from build123d import *

# Parameters (mm, degrees)
SKETCH_2_W          = 165
SKETCH_2_H          = 130
EXTRUDE_1_DEPTH     = 10
SKETCH_3_W          = 116
SKETCH_3_H          = 10
CUT_EXTRUDE_1_DEPTH = 10
CUT_EXTRUDE_2_DEPTH = 106.50473923
CHAMFER_1_SIZE      = 35
HOLE_WIZARD_M6_1_D  = 5
CHAMFER_3_SIZE      = 3


with BuildPart() as part:
    # 草图2 → 凸台-拉伸1 (new body)
    with BuildSketch(Plane(origin=(0, 0, 0), x_dir=(1, 0, 0), z_dir=(0, 1, 0))):
        Rectangle(SKETCH_2_W, SKETCH_2_H)
    extrude(amount=EXTRUDE_1_DEPTH)

    # 草图3 → 切除-拉伸1 (cut)
    with BuildSketch(Plane(origin=(0, 10, 0), x_dir=(1, 0, 0), z_dir=(0, 1, 0))):
        with Locations((0, 60)):
            Rectangle(SKETCH_3_W, SKETCH_3_H)
    extrude(amount=-CUT_EXTRUDE_1_DEPTH, mode=Mode.SUBTRACT)

    # 草图4 → 切除-拉伸2 (cut, through all)
    with BuildSketch(Plane(origin=(0, 10, 0), x_dir=(1, 0, 0), z_dir=(0, 1, 0))):
        with BuildLine():
            Line((75, 57.5), (75, 32.5))
            ThreePointArc((75, 32.5), (70.5, 28), (66, 32.5))
            Line((66, 32.5), (66, 57.5))
            ThreePointArc((66, 57.5), (70.5, 62), (75, 57.5))
        make_face()
        with BuildLine():
            Line((75, 17.5), (75, -7.5))
            ThreePointArc((75, -7.5), (70.5, -12), (66, -7.5))
            Line((66, -7.5), (66, 17.5))
            ThreePointArc((66, 17.5), (70.5, 22), (75, 17.5))
        make_face()
    cut_extrude_2 = extrude(amount=-CUT_EXTRUDE_2_DEPTH, mode=Mode.SUBTRACT)

    # 倒角1
    chamfer_1_edges = [part.edges().sort_by_distance(p)[0] for p in [
        (82.5, 5, 65),
        (-82.5, 5, 65),
    ]]
    chamfer(chamfer_1_edges, length=CHAMFER_1_SIZE)

    # M6 螺纹孔1 (through all)
    with Locations(Plane(origin=(0, 10, 0), x_dir=(1, 0, 0), z_dir=(0, 1, 0))):
        with Locations((21, -14), (21, 34), (-21, 34), (-21, -14)):
            Hole(HOLE_WIZARD_M6_1_D / 2)

    # 倒角3
    chamfer_3_edges = [part.edges().sort_by_distance(p)[0] for p in [
        (-82.5, 5, -65),
        (82.5, 5, -65),
    ]]
    chamfer(chamfer_3_edges, length=CHAMFER_3_SIZE)

    # 镜向1: 切除-拉伸2 across plane
    add(cut_extrude_2.mirror(Plane(origin=(0, 0, 0), x_dir=(0, 0, 1), z_dir=(1, 0, 0))), mode=Mode.SUBTRACT)


solid = part.part
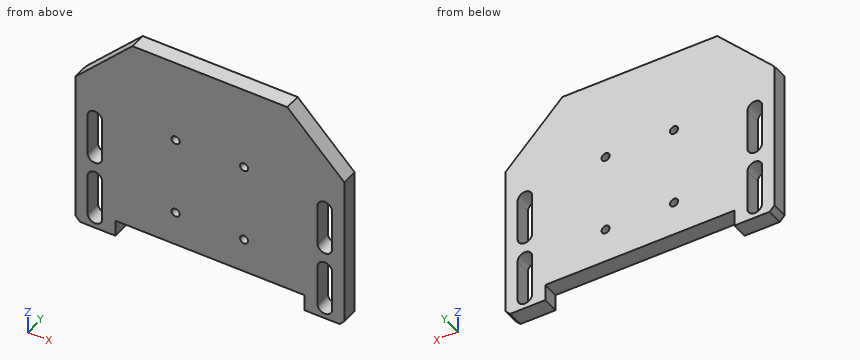
Work out the finished part from the listing and answer in its coordinate system (mm). Coordinates: 2 decimals unless noted, no trailing zeros. Loops run counter-clockwise (first coordinate to the right, second up) from the corner with the lowest first, then second, coordinate; pieces in that order, holes last. Notation, with made-up numbers: (13, 87.5) -> (68, 87.5) arc R11 cw to (68, 94.5) -> close; hole circle Ø4 at (-19.5, -1). An arc over 180 degrees is marked (long way). Write each question's results on one line, items separated by ' | '. Start each with the question number.
1) Find section C-C on y = 1.75. Count the separate pieces of the cut face and the enclosed holes in it, then the cut area to 3 significant figures.
2) Find section A-A on z = -5.5. Determine the outline of the cut face in (x, y).
3) Find section D-D on z = 37. Determine the outline of the cut face in (x, y), then the cut area to 3 significant figures.
4) Flat-ended cylindrical pins translate along their axes: P1, Ø6, axis at x = 21, z = 14, coming from the -Y side; P2, Ø6, axis at y = 6.5, z = 44, coming from the -X side. Find the tip coordinate at first contact, or state that the pin passes through.
5) Find section B-B on x = 21. Determine the outline of the cut face in (y, z), then the cut area to 3 significant figures.
6) Consider line 1 along X through (y, z) = (2.75, 14); line 2 along Z through (x, y) = (-21, 3.5); line 3 along X through (y, z) = (6, -16.5). Determine where each line is inside the solid, lowest interval first.
Response values:
1) separate pieces: 1 | enclosed holes: 8 | area: 17,800 mm^2
2) outline: (-82.5, 0) -> (-75, 0) -> (-75, 10) -> (-82.5, 10) -> close; (-66, 0) -> (66, 0) -> (66, 10) -> (-66, 10) -> close; (75, 0) -> (82.5, 0) -> (82.5, 10) -> (75, 10) -> close
3) outline: (-75.5, 0) -> (75.5, 0) -> (75.5, 10) -> (-75.5, 10) -> close | area: 1,510 mm^2
4) P1: stops at y = 0 | P2: stops at x = -71.5
5) outline: (0, -55) -> (10, -55) -> (10, -36.5) -> (0, -36.5) -> close; (0, -31.5) -> (10, -31.5) -> (10, 11.5) -> (0, 11.5) -> close; (0, 16.5) -> (10, 16.5) -> (10, 65) -> (0, 65) -> close | area: 1,100 mm^2
6) line 1: x = -82.5 to -23.5, -18.5 to 18.5, 23.5 to 82.5 | line 2: z = -55 to -36.5, -31.5 to 11.5, 16.5 to 65 | line 3: x = -82.5 to -75, -66 to 66, 75 to 82.5
